Part model, mm, in its own coordinate system. Give positions to 0.01 mm unless a question says otherwise; leave off trailing zeros. Write each loop counter-clockwise with the first axis right and the second up, starting at its lowest first coordinate (ties: lowest second). Pieces come first, ordered by that corner, then holes.
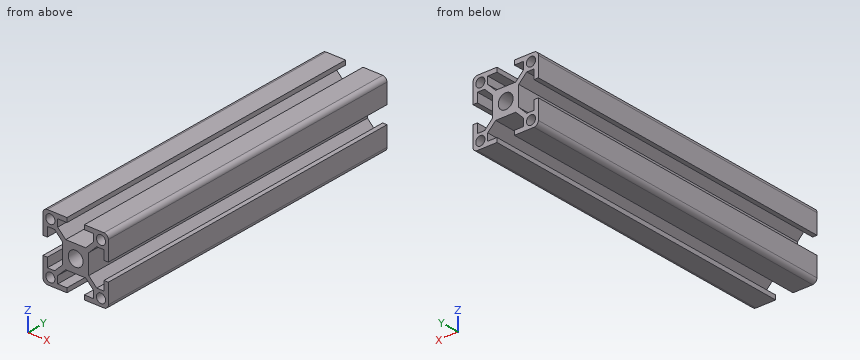
from build123d import *

# Parameters (mm, degrees)
SKETCH_1_R      = 2.1
SKETCH_1_R_2    = 3.4
EXTRUDE_1_DEPTH = 150


with BuildPart() as part:
    # 草图1 → 拉伸1 (new body)
    with BuildSketch(Plane(origin=(0, 0, 0), x_dir=(1, 0, 0), z_dir=(0, 1, 0))):
        with BuildLine():
            Line((6.75, -28), (11, -28))
            Line((11, -28), (11, -30))
            Line((11, -30), (2, -30))
            ThreePointArc((2, -30), (0.585786438, -29.414213562), (0, -28))
            Line((0, -28), (0, -19))
            Line((0, -19), (2, -19))
            Line((2, -19), (2, -23.25))
            Line((2, -23.25), (5.335785999, -23.25))
            Line((5.335785999, -23.25), (9, -19.585785999))
            Line((9, -19.585785999), (9, -10.414214001))
            Line((9, -10.414214001), (5.335785999, -6.75))
            Line((5.335785999, -6.75), (2, -6.75))
            Line((2, -6.75), (2, -11))
            Line((2, -11), (0, -11))
            Line((0, -11), (0, -2))
            ThreePointArc((0, -2), (0.585786438, -0.585786438), (2, 0))
            Line((2, 0), (11, 0))
            Line((11, 0), (11, -2))
            Line((11, -2), (6.75, -2))
            Line((6.75, -2), (6.75, -5.335785999))
            Line((6.75, -5.335785999), (10.414214001, -9))
            Line((10.414214001, -9), (19.585785999, -9))
            Line((19.585785999, -9), (23.25, -5.335785999))
            Line((23.25, -5.335785999), (23.25, -2))
            Line((23.25, -2), (19, -2))
            Line((19, -2), (19, 0))
            Line((19, 0), (28, 0))
            ThreePointArc((28, 0), (29.414213562, -0.585786438), (30, -2))
            Line((30, -2), (30, -11))
            Line((30, -11), (28, -11))
            Line((28, -11), (28, -6.75))
            Line((28, -6.75), (24.664214001, -6.75))
            Line((24.664214001, -6.75), (21, -10.414214001))
            Line((21, -10.414214001), (21, -19.585785999))
            Line((21, -19.585785999), (24.664214001, -23.25))
            Line((24.664214001, -23.25), (28, -23.25))
            Line((28, -23.25), (28, -19))
            Line((28, -19), (30, -19))
            Line((30, -19), (30, -28))
            ThreePointArc((30, -28), (29.414213562, -29.414213562), (28, -30))
            Line((28, -30), (19, -30))
            Line((19, -30), (19, -28))
            Line((19, -28), (23.25, -28))
            Line((23.25, -28), (23.25, -24.664214001))
            Line((23.25, -24.664214001), (19.585785999, -21))
            Line((19.585785999, -21), (10.414214001, -21))
            Line((10.414214001, -21), (6.75, -24.664214001))
            Line((6.75, -24.664214001), (6.75, -28))
        make_face()
        with Locations(Location((3.375, -26.625, 0), (0, 0, 270))):
            Circle(SKETCH_1_R, mode=Mode.SUBTRACT)
        with Locations(Location((26.625, -26.625, 0), (0, 0, 270))):
            Circle(SKETCH_1_R, mode=Mode.SUBTRACT)
        with Locations(Location((15, -15, 0), (0, 0, 270))):
            Circle(SKETCH_1_R_2, mode=Mode.SUBTRACT)
        with Locations(Location((3.375, -3.375, 0), (0, 0, 270))):
            Circle(SKETCH_1_R, mode=Mode.SUBTRACT)
        with Locations(Location((26.625, -3.375, 0), (0, 0, 270))):
            Circle(SKETCH_1_R, mode=Mode.SUBTRACT)
    extrude(amount=EXTRUDE_1_DEPTH)


solid = part.part
1) Saw through at C-C (y = 118). State how many separate pieces and enclosed holes the cut face has, and give its area (3 significant figures).
Check result:
separate pieces: 1
enclosed holes: 5
area: 333 mm2
2) Flat gauge pins, fed straight in: P1, Ø4.5, axis at y = 88, z = 15, coming from the +X side; P2, Ø1, axis at y = 20.5, z = 17, coming from the -X side; P3, Ø1, axis at y = 69.5, z = 1, coming from the -X side; P4, Ø2.5, axis at x = 26.625, z = 3.375, coming from the -Y side. Where does each tip first touch, or does it go through?
Check result:
P1: stops at x = 21
P2: stops at x = 9
P3: stops at x = 0.06
P4: passes through
3) Saw through at A-A (z = 15). Write the cut outline in (x, y), and give its area (3 significant figures).
Check result:
outline: (9, 0) - (11.6, 0) - (11.6, 150) - (9, 150) - close; (18.4, 0) - (21, 0) - (21, 150) - (18.4, 150) - close
area: 780 mm2
4) Drill centre lines: L1, parallel to X at y = 125, z = 26.75; L2, parallel to X at y = 95, z = 27.25; L3, parallel to Z at x = 22.75, y = 128.5. Where is each one in solid material? Low to high.
Check result:
L1: x = 0 to 1.28, 5.47 to 6.75, 23.25 to 24.53, 28.72 to 30
L2: x = 0 to 1.37, 5.38 to 6.75, 23.25 to 24.62, 28.63 to 30
L3: z = 0 to 2, 5.84 to 8.66, 21.34 to 24.16, 28 to 30
5) Saw through at B-B (x = 15). Write the cut outline in (y, z), and give its area (3 significant figures).
Check result:
outline: (0, 9) - (150, 9) - (150, 11.6) - (0, 11.6) - close; (0, 18.4) - (150, 18.4) - (150, 21) - (0, 21) - close
area: 780 mm2
